The model under review builds one solid part; all positions refer to its coordinate system, in mm. Face numbers are marked on the shaded views. Coordinates: 2 decimals unless noted, no trailing zeros. Loops run counter-clockwise (first coordinate to the right, second up) from the corner with the lowest first, then second, coordinate; pieces in that order, holes last. Notation, with made-up numbers: M -10.5,68.25 L 24.5,68.25 A18 ccw 24.5,96.25 Z; hole C -32.75,36.5 d10. An arc over 180 degrees is marked long. Write item = value, one per line. Start each with the question number.
Q1. Mouldability with a two-part tool opening along X and no side actions: class the marked faces 1, 2, 3 and 4 as released by +X, released by -X, zero draft, split by the parting line, or undercut.
Q2. Clearance check with flat-ended pins moving along their axes: pin 1 Ø6 at (y, z) = (5, 7) entering from +X; pin 2 Ø5 at (y, z) = (6.5, 6.5) entering from +X; pin 3 Ø1.5 at (y, z) = (4, 6) entering from +X. State where each tip first meets the part, or that it passes through.
Q3. Wall thickness on probe 1 along Y at (x, z) = (0, 3.65); probe 2 along Y at (x, z) = (-3.25, 1.5); probe 3 along X at (y, z) = (4, 1): over which ranges is each line inside the solid? List them lowest first.
Q4. We need section D-D on z = 8.5. Give the boundary of the cut face in (x, y), and give its area (3 significant figures).
Q5. We need section A-A on x = 0. Give the boundary of the cut face in (y, z).
Q6. We need section C-C on z = 3.5. Give the boundary of the cut face in (x, y), and give its area (3 significant figures).
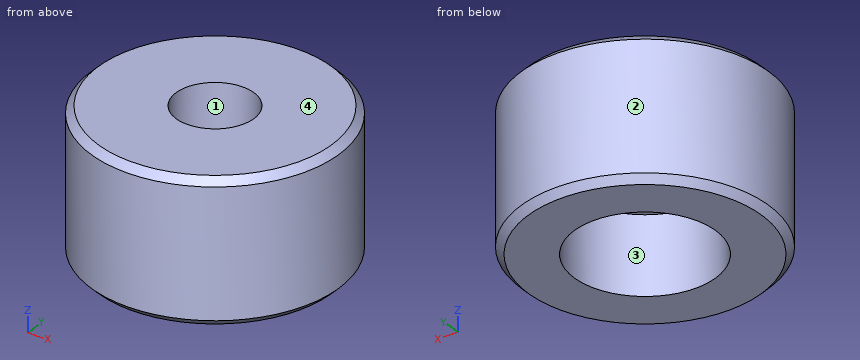
from build123d import *

# Parameters (mm, degrees)
SKETCH1_R           = 8.75
SKETCH1_R_2         = 2.75
BOSS_EXTRUDE1_DEPTH = 10
SKETCH2_R           = 5
CUT_EXTRUDE1_DEPTH  = 5.5
CHAMFER1_SIZE       = 0.5


with BuildPart() as part:
    # Sketch1 → Boss-Extrude1 (new body)
    with BuildSketch(Plane.XY):
        Circle(SKETCH1_R)
        Circle(SKETCH1_R_2, mode=Mode.SUBTRACT)
    extrude(amount=BOSS_EXTRUDE1_DEPTH)

    # Sketch2 → Cut-Extrude1 (cut)
    with BuildSketch(Plane(origin=(0, 0, 0), x_dir=(-1, 0, 0), z_dir=(0, 0, -1))):
        Circle(SKETCH2_R)
    extrude(amount=-CUT_EXTRUDE1_DEPTH, mode=Mode.SUBTRACT)

    # Chamfer1
    chamfer1_edges = [part.edges().sort_by_distance(p)[0] for p in [
        (-8.75, 0, 0),
        (-8.75, 0, 10),
    ]]
    chamfer(chamfer1_edges, length=CHAMFER1_SIZE)


solid = part.part
Returned:
q1.face_1 = undercut
q1.face_2 = split by the parting line
q1.face_3 = undercut
q1.face_4 = zero draft
q2.pin_1 = 8.52
q2.pin_2 = 7.78
q2.pin_3 = 8.12
q3.probe_1 = -8.75 to -5, 5 to 8.75
q3.probe_2 = -8.12 to -3.8, 3.8 to 8.12
q3.probe_3 = -7.78 to -3, 3 to 7.78
q4.outline = C 0,0 d17.5; hole C 0,0 d5.5
q4.area = 217 mm^2
q5.outline = M -8.75,0.5 L -8.25,0 L -5,0 L -5,5.5 L -2.75,5.5 L -2.75,10 L -8.25,10 L -8.75,9.5 Z; M 2.75,5.5 L 5,5.5 L 5,0 L 8.25,0 L 8.75,0.5 L 8.75,9.5 L 8.25,10 L 2.75,10 Z
q6.outline = C 0,0 d17.5; hole C 0,0 d10
q6.area = 162 mm^2
